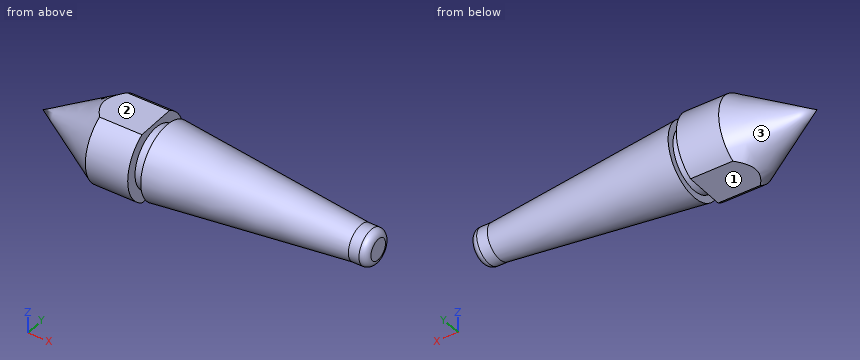
```python
from build123d import *

# Parameters (mm, degrees)
FILLET1_R          = 2
CUT_EXTRUDE1_DEPTH = 66.065351763


with BuildPart() as part:
    # Sketch1 → Revolve1 (revolve)
    with BuildSketch(Plane.XY, mode=Mode.PRIVATE) as revolve1_sk:
        Polygon((0, 0), (0, 5), (-5, 5), (-60, 10.5), (-60, 8.5), (-63, 8.5), (-63, 11.5), (-75, 11.5), (-94.92, 0), align=None)
    revolve(revolve1_sk.sketch.rotate(Axis((-94.92, 0, 0), (1, 0, 0)), 90), axis=Axis((-94.92, 0, 0), (1, 0, 0)))

    # Fillet1
    fillet1_edges = [part.edges().sort_by_distance(p)[0] for p in [
        (0, 0, -5),
    ]]
    fillet(fillet1_edges, radius=FILLET1_R)

    # Sketch2 → Cut-Extrude1 (cut, through all)
    with BuildSketch(Plane(origin=(-63, 0, 0), x_dir=(0, 0, -1), z_dir=(1, 0, 0))):
        with BuildLine():
            Line((-10, 5.678908346), (-10, -5.678908346))
            ThreePointArc((-10, -5.678908346), (-11.5, 0), (-10, 5.678908346))
        make_face()
        with BuildLine():
            Line((10, 5.678908346), (10, -5.678908346))
            ThreePointArc((10, -5.678908346), (11.5, 0), (10, 5.678908346))
        make_face()
    extrude(amount=-CUT_EXTRUDE1_DEPTH, mode=Mode.SUBTRACT)


solid = part.part
```
CAD build for the part. Positions are in the model's coordinates, mm. Face numbers are marked on the shaded views. A direction names the side the tool comes from. Coordinates: 2 decimals unless noted, no trailing zeros. Order: outer loops, then holes, each group sorted by start corner. A loop starts at its lowest first (then second) coordinate and runs counter-clockwise, first axis right, second up.
(1) Which spindle directions (+Z, -Z, +X, -X, +Y, -Y) get a long thin tool onto all of the face, cutting with end or side? Do the marked faces 1, 2 and 3. Say none if no direction does.
Solution:
face 1: -Z, -X, +Y, -Y
face 2: +Z, -X, +Y, -Y
face 3: -X
(2) Saw through at C-C, the plane x = -37. Write the cut outline in (y, z).
Solution:
outline: circle Ø16.4 at (0, 0)
(3) Drill centre lines: L1, parallel to Y at x = -64, z = 1.25; L2, parallel to Y at x = -40, z = -7; L3, parallel to Z at x = -66, y = -7. Where is each one in solid material? Low to high.
Solution:
L1: y = -11.43 to 11.43
L2: y = -4.82 to 4.82
L3: z = -9.12 to 9.12
(4) Pin check, flat tips, straight feed: pin 1 Ø6 at (y, z) = (4.5, -4.5) entering from -X; pin 2 Ø4 at (x, y) = (-53, 6.5) entering from -Z; pin 3 Ø12.5 at (x, y) = (-70, -0.5) entering from -Z; pin 4 Ø6 at (y, z) = (-1, 3.5) entering from +X. Stop position of each tip, or through.
Solution:
pin 1: stops at x = -89.09
pin 2: stops at z = -8.73
pin 3: stops at z = -10
pin 4: stops at x = 0
(5) Saw through at B-B, the plane x = -72. Write the cut outline in (y, z).
Solution:
outline: (-5.68, -10) - (5.68, -10) arc R11.5 ccw to (5.68, 10) - (-5.68, 10) arc R11.5 ccw to start
(6) Saw through at A-A, the plane x = -55.5. Write the cut outline in (y, z).
Solution:
outline: circle Ø20.1 at (0, 0)
